Could you check a few things on this model? Use its own coordinates, in mm. Face numbers are marked on the shaded views. A direction names the side the tool comes from. Coordinates: 2 decimals unless noted, no trailing zeros. Order: outer loops, then holes, each group sorted by start corner. A loop starts at its lowest first (then second) coordinate and runs counter-clockwise, first axis right, second up. Notation, with made-up numbers: (13.5, 56.25) - (26.5, 56.25) arc R18 ccw to (26.5, 82.25) - close; hole circle Ø2 at (20.5, 38.5). An arc over 180 degrees is marked (long way). One line per item, written item: value.
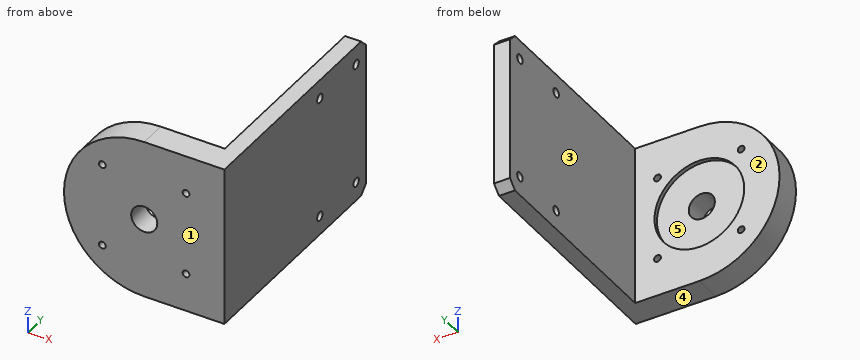
from build123d import *

# Parameters (mm, degrees)
BOSS_EXTRUDE1_DEPTH = 29.5
SKETCH2_R           = 4.8
CUT_EXTRUDE1_DEPTH  = 10
SKETCH4_R           = 16.5
CUT_EXTRUDE2_DEPTH  = 1.5
M3_TAPPED_HOLE1_D   = 2.5
CHAMFER1_SIZE       = 3
M4_TAPPED_HOLE1_D   = 3.3


with BuildPart() as part:
    # Sketch1 → Boss-Extrude1 (new, symmetric)
    with BuildSketch(Plane.XY):
        Polygon((15.9, 0.233022363), (-43.1, 0.233022363), (-43.1, 10.233022363), (10, 10.233022363), (10, 86.233022363), (15.9, 86.233022363), align=None)
    extrude(amount=BOSS_EXTRUDE1_DEPTH, both=True)

    # Sketch2 → Cut-Extrude1 (cut)
    with BuildSketch(Plane.XZ.offset(-0.233022363)):
        with BuildLine():
            ThreePointArc((-43.1, 0), (-34.459650045, 20.859650045), (-13.6, 29.5))
            Line((-13.6, 29.5), (-43.1, 29.5))
            Line((-43.1, 29.5), (-43.1, 0))
        make_face()
        with BuildLine():
            ThreePointArc((-13.6, -29.5), (-34.459650045, -20.859650045), (-43.1, 0))
            Line((-43.1, 0), (-43.1, -29.5))
            Line((-43.1, -29.5), (-13.6, -29.5))
        make_face()
        with Locations((-13.6, 0)):
            Circle(SKETCH2_R)
    extrude(amount=-CUT_EXTRUDE1_DEPTH, mode=Mode.SUBTRACT)

    # Sketch4 → Cut-Extrude2 (cut)
    with BuildSketch(Plane(origin=(0, 10.233022363, 0), x_dir=(1, 0, 0), z_dir=(0, 1, 0))):
        with Locations(Location((-13.6, 0, 0), (0, 0, 180))):
            Circle(SKETCH4_R)
    extrude(amount=-CUT_EXTRUDE2_DEPTH, mode=Mode.SUBTRACT)

    # M3 Tapped Hole1 (through all)
    with Locations(Plane(origin=(0, 10.233022363, 0), x_dir=(1, 0, 0), z_dir=(0, 1, 0))):
        with Locations((-28.979572491, -15.379572491), (-28.979572491, 15.379572491), (1.779572491, 15.379572491), (1.779572491, -15.379572491)):
            Hole(M3_TAPPED_HOLE1_D / 2)

    # Chamfer1
    chamfer1_edges = [part.edges().sort_by_distance(p)[0] for p in [
        (12.95, 86.233022363, 29.5),
        (12.95, 86.233022363, -29.5),
    ]]
    chamfer(chamfer1_edges, length=CHAMFER1_SIZE)

    # M4 Tapped Hole1 (through all)
    with Locations(Plane.ZY.offset(-10)):
        with Locations((-22.5, 80.233022363), (-22.5, 58.233022363), (22.5, 58.233022363), (22.5, 80.233022363)):
            Hole(M4_TAPPED_HOLE1_D / 2)


solid = part.part
Item 1: If I drill on probe 1 along X at (y, z) = (71, -14.5); probe 2 along Y at (x, z) = (-24.5, 13); probe 3 along Y at (x, z) = (-18.5, 11), over which ranges is the centre line in solid material (lowest first)?
Conclusion:
probe 1: 10 to 15.9
probe 2: 0.23 to 10.23
probe 3: 0.23 to 8.73
Item 2: Thinking about a two-plate mould opening in Z: for the marked faces 3, 4 and 5, which applies, pulls with the +Z half, pulls with the -Z half, needs draft (parallel to the pull), parting line crosses it, or undercut?
Conclusion:
face 3: needs draft
face 4: pulls with the -Z half
face 5: undercut
Item 3: I want a section at C-C on y = 46. Please give me the cut outline in (x, z), then the cut area to 3 significant figures.
Conclusion:
outline: (10, -29.5) - (15.9, -29.5) - (15.9, 29.5) - (10, 29.5) - close
area: 348 mm²
Item 4: I want a section at B-B on x = -11.5. Please give me the cut outline in (y, z), then the cut area to 3 significant figures.
Conclusion:
outline: (0.23, -29.5) - (10.23, -29.5) - (10.23, -16.37) - (8.73, -16.37) - (8.73, -4.32) - (0.23, -4.32) - close; (0.23, 4.32) - (8.73, 4.32) - (8.73, 16.37) - (10.23, 16.37) - (10.23, 29.5) - (0.23, 29.5) - close
area: 468 mm²
Item 5: I want a section at D-D on z = -22.5. Please give me the cut outline in (x, y).
Conclusion:
outline: (-32.68, 0.23) - (15.9, 0.23) - (15.9, 56.58) - (10, 56.58) - (10, 10.23) - (-32.68, 10.23) - close; (10, 59.88) - (15.9, 59.88) - (15.9, 78.58) - (10, 78.58) - close; (10, 81.88) - (15.9, 81.88) - (15.9, 86.23) - (10, 86.23) - close
Item 6: I'm going to push flat-ended pins straight in: pin 1 Ø5 at (x, y) = (-17, 12) entering from +Z; pin 2 Ø1 at (x, z) = (-29.5, -9.5) entering from +Y; pin 3 Ø4 at (y, z) = (80.23, -22.5) entering from -X. Where does each tip first touch, or does it pass through?
Conclusion:
pin 1: z = 29.45
pin 2: y = 10.23
pin 3: x = 10
Item 7: For the marked faces 1 and 2, which set-ups out of +Z, -Z, +X, -X, +Y, -Y let a thin tool reach every point of the face, with its end or its side?
Conclusion:
face 1: +Z, -Z, +X, -X, -Y
face 2: +Z, -Z, -X, +Y
Item 8: I want a section at A-A on z = 0. Please give me the cut outline in (x, y).
Conclusion:
outline: (-43.1, 0.23) - (-18.4, 0.23) - (-18.4, 8.73) - (-30.1, 8.73) - (-30.1, 10.23) - (-43.1, 10.23) - close; (-8.8, 0.23) - (15.9, 0.23) - (15.9, 86.23) - (10, 86.23) - (10, 10.23) - (2.9, 10.23) - (2.9, 8.73) - (-8.8, 8.73) - close
